from build123d import *

# Parameters (mm, degrees)
SKETCH_1_W         = 70
SKETCH_1_H         = 70
EXTRUDE_1_DEPTH    = 32
SKETCH_2_R         = 35
EXTRUDE_2_DEPTH    = 80
FILLET_1_R         = 6
FILLET_2_R         = 5
SKETCH_3_R         = 5
EXTRUDE_3_DEPTH    = 32
HOLE_WIZARD_M5_1_D = 4.2
SKETCH_7_R         = 12
EXTRUDE_4_DEPTH    = 3


with BuildPart() as part:
    # 草图1 → 凸台-拉伸1 (new body)
    with BuildSketch(Plane.XY):
        Rectangle(SKETCH_1_W, SKETCH_1_H)
    extrude(amount=EXTRUDE_1_DEPTH)

    # 草图2 → 凸台-拉伸2 (add)
    with BuildSketch(Plane(origin=(0, 0, 0), x_dir=(-1, 0, 0), z_dir=(0, 0, -1))):
        Circle(SKETCH_2_R)
    extrude(amount=EXTRUDE_2_DEPTH)

    # 圆角1
    fillet_1_edges = [part.edges().sort_by_distance(p)[0] for p in [
        (35, -35, 16),
        (-35, -35, 16),
        (-35, 35, 16),
        (35, 35, 16),
    ]]
    fillet(fillet_1_edges, radius=FILLET_1_R)

    # 圆角2
    fillet_2_edges = [part.edges().sort_by_distance(p)[0] for p in [
        (35, 0, -80),
    ]]
    fillet(fillet_2_edges, radius=FILLET_2_R)

    # 草图3 → 凸台-拉伸3 (add)
    with BuildSketch(Plane.XY.offset(32)):
        with Locations((0, 15)):
            Circle(SKETCH_3_R)
    extrude(amount=EXTRUDE_3_DEPTH)

    # M5 螺纹孔1 (through all)
    with Locations(Plane.XY.offset(32)):
        with Locations((-28.991378029, 28.991378029), (-28.991378029, -28.991378029), (28.991378029, -28.991378029), (28.991378029, 28.991378029)):
            Hole(HOLE_WIZARD_M5_1_D / 2)

    # 草图7 → 凸台-拉伸4 (add)
    with BuildSketch(Plane.XY.offset(32)):
        with Locations((0, 15)):
            Circle(SKETCH_7_R)
    extrude(amount=EXTRUDE_4_DEPTH)


solid = part.part
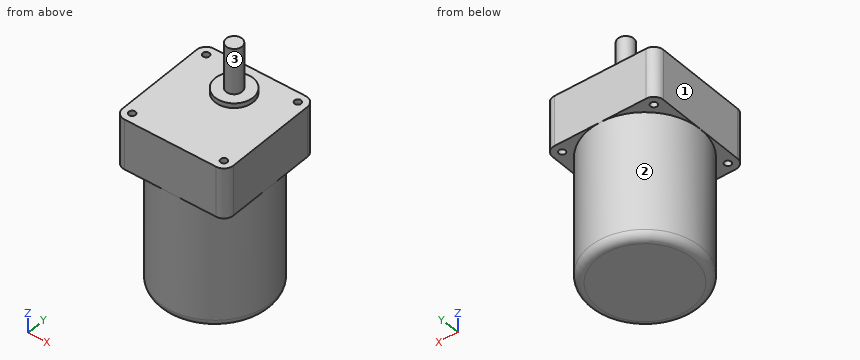
Design review of the part built by this model. Coordinates are the model's own, in mm. Face numbers are marked on the shaded views. A direction names the side the tool comes from. Coordinates: 2 decimals unless noted, no trailing zeros.
Item 1: For the marked faces 1, 2 and 3, list the 3-axis set-ups (+Z, -Z, +X, -X, +Y, -Y) from which the entire face can be reached by the end or side of a thin tool; tool diameter is ignored.
Item 2: For line 1 (X direction, y = -30, z = 13.5); line 2 (Z direction, x = -22, y = -20); line 3 (Z direction, x = 27, y = 31), list the stretches that pass through material, from the lowest coordinate up.
Item 3: For pin 1 Ø3 at (x, y) = (20, 14) entering from +Z; pin 2 Ø2 at (y, z) = (-2.5, -0.5) entering from +X; pin 3 Ø2.5 at (x, y) = (-28.99, 28.99) entering from +Z; pin 4 Ø6 at (y, z) = (11.5, -42) entering from -X, all flat-tipped, find the tip position at first contact; note any pin that passes through.
The answers:
1. face 1: +Z, -Z, -X, +Y, -Y
1. face 2: -Z
1. face 3: +Z
2. line 1: x = -34.92 to -30.83, -27.15 to 27.15, 30.83 to 34.92
2. line 2: z = -80 to 32
2. line 3: z = 0 to 32
3. pin 1: stops at z = 32
3. pin 2: stops at x = 35
3. pin 3: passes through
3. pin 4: stops at x = -33.95
